Source: CAD feature listing. Evaluate the final solid. Frame: model axes, mm. Face numbers are marked on the shaded views. Round coordinates to 2 decimals unless told otherwise and drop trailing zeros. Loops run counter-clockwise (first coordinate to the right, second up) from the corner with the lowest first, then second, coordinate; pieces in that order, holes last. Notation, with made-up numbers: M 65,13.5 L 80,13.5 A25 cw 80,31.5 Z; hole C 49.25,50 d6. An arc over 180 degrees is marked long. Answer as CSV lines item,"result". Start each with the question number.
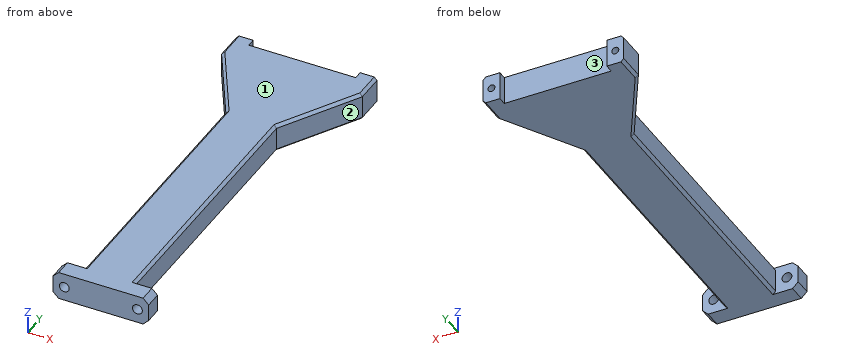
```python
from build123d import *

# Parameters (mm, degrees)
SKETCH1_W                      = 50
SKETCH1_H                      = 140
BOSS_EXTRUDE1_DEPTH            = 5
CUT_EXTRUDE1_DEPTH             = 76
SKETCH3_W                      = 38
SKETCH3_H                      = 3
CUT_EXTRUDE2_DEPTH             = 76
M3_TAPPED_HOLE1_D              = 2.5
M3_TAPPED_HOLE1_DEPTH          = 8.5
M3_TAPPED_HOLE1_TIP            = 0.751075774
F_3_5_3_5_DIAMETER_HOLE1_D     = 3.5
F_3_5_3_5_DIAMETER_HOLE1_DEPTH = 6
CHAMFER1_SIZE                  = 2
CHAMFER2_SIZE                  = 1


with BuildPart() as part:
    # Sketch1 → Boss-Extrude1 (new, symmetric)
    with BuildSketch(Plane.XY):
        Rectangle(SKETCH1_W, SKETCH1_H)
    extrude(amount=BOSS_EXTRUDE1_DEPTH, both=True)

    # Sketch2 → Cut-Extrude1 (cut, through all)
    with BuildSketch(Plane.XY.offset(5)):
        Polygon((-25, 60), (-9, 32.287187079), (-9, -64), (-17, -64), (-17, -70), (-25, -70), align=None)
    cut_extrude1 = extrude(amount=-CUT_EXTRUDE1_DEPTH, mode=Mode.SUBTRACT)

    # Mirror1: Cut-Extrude1 across plane
    add(cut_extrude1.mirror(Plane(origin=(0, 0, 0), x_dir=(0, 0, 1), z_dir=(1, 0, 0))), mode=Mode.SUBTRACT)

    # Sketch3 → Cut-Extrude2 (cut, through all)
    with BuildSketch(Plane.XY.offset(5)):
        with Locations((0, 68.5)):
            Rectangle(SKETCH3_W, SKETCH3_H)
    extrude(amount=-CUT_EXTRUDE2_DEPTH, mode=Mode.SUBTRACT)

    # M3 Tapped Hole1
    with Locations(Plane(origin=(0, 70, 0), x_dir=(1, 0, 0), z_dir=(0, 1, 0))):
        with Locations((-22, 0), (22, 0)):
            Hole(M3_TAPPED_HOLE1_D / 2, depth=M3_TAPPED_HOLE1_DEPTH)
            with Locations((0, 0, -(M3_TAPPED_HOLE1_DEPTH + M3_TAPPED_HOLE1_TIP / 2))):  # 118° drill point
                Cone(0, M3_TAPPED_HOLE1_D / 2, M3_TAPPED_HOLE1_TIP, mode=Mode.SUBTRACT)

    # Ø3.5 (3.5) Diameter Hole1
    with Locations(Plane(origin=(0, -70, 0), x_dir=(-1, 0, 0), z_dir=(0, -1, 0))):
        with Locations((13, 0), (-13, 0)):
            Hole(F_3_5_3_5_DIAMETER_HOLE1_D / 2, depth=F_3_5_3_5_DIAMETER_HOLE1_DEPTH)

    # Chamfer1
    chamfer1_edges = [part.edges().sort_by_distance(p)[0] for p in [
        (-17, -67, -5),
        (-17, -67, 5),
        (17, -67, 5),
        (17, -67, -5),
    ]]
    chamfer(chamfer1_edges, length=CHAMFER1_SIZE)

    # Chamfer2
    chamfer2_edges = [part.edges().sort_by_distance(p)[0] for p in [
        (-25, 65, 5),
        (-17, 46.143593539, -5),
        (-9, -15.856406461, -5),
        (-9, -15.856406461, 5),
        (-17, 46.143593539, 5),
        (25, 65, -5),
        (25, 65, 5),
        (9, -15.856406461, 5),
        (17, 46.143593539, 5),
        (9, -15.856406461, -5),
        (17, 46.143593539, -5),
        (-25, 65, -5),
    ]]
    chamfer(chamfer2_edges, length=CHAMFER2_SIZE)


solid = part.part
```
1) Mould query, pull axis X, two halves, no side actions, for the marked faces 1, 2 and 3. Classes: pulls with the +X half, pulls with the -X half, needs draft (parallel to the pull), parting line crosses it, or undercut.
2) Ray query, line 1 along Z through (x, y) = (22, 68); line 2 along X through (y, z) = (9, 0); line 3 along Y through (x, z) = (2, -2). Return the intervals inside material, ascending.
3) Section B-B, the plane y = 31. Return loops of the section in (x, z), and give its area (3 significant figures).
4) Contact query for flat-ended pins moving along their axis: pin 1 Ø2 at (x, z) = (-22, 0) entering from +Y; pin 2 Ø2.5 at (y, z) = (7, -0.5) entering from +X; pin 3 Ø5 at (y, z) = (-68, 1) entering from +X. Output: stop coordinate, or through.
5) Section A-A, the plane x = 13. Return loops of the section in (y, z), and give its area (3 significant figures).
6) Section C-C, the plane y = 52.5. Return loops of the section in (x, z), and give its area (3 significant figures).
Findings below:
1,face 1,"needs draft"
1,face 2,"pulls with the +X half"
1,face 3,"undercut"
2,line 1,"-5 to -1.25, 1.25 to 5"
2,line 2,"-9 to 9"
2,line 3,"-70 to 67"
3,outline,"M -9,-4 L -8,-5 L 8,-5 L 9,-4 L 9,4 L 8,5 L -8,5 L -9,4 Z"
3,area,"178 mm²"
4,pin 1,"y = 61.35"
4,pin 2,"x = 9"
4,pin 3,"x = 17"
5,outline,"M -70,-5 L -64,-5 L -64,-1.75 L -70,-1.75 Z; M -70,1.75 L -64,1.75 L -64,5 L -70,5 Z; M 39.22,-4 L 41.22,-5 L 67,-5 L 67,5 L 41.22,5 L 39.22,4 Z"
5,area,"315 mm²"
6,outline,"M -20.67,-4 L -19.52,-5 L 19.52,-5 L 20.67,-4 L 20.67,4 L 19.52,5 L -19.52,5 L -20.67,4 Z"
6,area,"411 mm²"
